Source: CAD feature listing. Evaluate the final solid. Frame: model axes, mm. Give positions to 0.01 mm unless a question says otherwise; leave off trailing zeros. Write each loop counter-clockwise with the first axis right and the second up, starting at its lowest first coordinate (ties: lowest second). Pieces come first, ordered by that corner, then holes. Notation, with made-up numbers: M 19.5,-12 L 78.5,-12 A23 cw 78.5,15 Z; hole C 17.25,43 d2. An arc over 180 degrees is marked long. Answer as a JSON object with one key per item and string values. Group by question number.
```python
from build123d import *

# Parameters (mm, degrees)
BASE_BLOCK_SKETCH_W         = 60
BASE_BLOCK_SKETCH_H         = 100
BASE_BLOCK_DEPTH            = 30
LOWER_CELL_POCKETS_SKETCH_W = 26
LOWER_CELL_POCKETS_SKETCH_H = 12
LOWER_CELL_POCKETS_DEPTH    = 66.574385243
UPPER_STEP_SKETCH_W         = 60
UPPER_STEP_SKETCH_H         = 57
UPPER_STEP_BOSS_DEPTH       = 20
UPPER_CELL_POCKETS_SKETCH_W = 26
UPPER_CELL_POCKETS_SKETCH_H = 16
UPPER_CELL_POCKETS_DEPTH    = 77.811457479
BACK_WALL_SLOTS_SKETCH_W    = 10.8
BACK_WALL_SLOTS_SKETCH_H    = 7
BACK_WALL_SLOTS_DEPTH       = 66.574385243


with BuildPart() as part:
    # Base Block Sketch → Base Block (new body)
    with BuildSketch(Plane.XY):
        Rectangle(BASE_BLOCK_SKETCH_W, BASE_BLOCK_SKETCH_H)
    extrude(amount=BASE_BLOCK_DEPTH)

    # Lower Cell Pockets Sketch → Lower Cell Pockets (cut, through all)
    with BuildSketch(Plane.XY.offset(30)):
        with Locations((14, 41)):
            Rectangle(LOWER_CELL_POCKETS_SKETCH_W, LOWER_CELL_POCKETS_SKETCH_H)
        Polygon((-21.788065722, 47), (-27, 47), (-27, 35), (-1, 35), (-1, 47), align=None)
    extrude(amount=-LOWER_CELL_POCKETS_DEPTH, mode=Mode.SUBTRACT)

    # Upper Step Sketch → Upper Step Boss (add)
    with BuildSketch(Plane.XY.offset(30)):
        with Locations((0, -21.5)):
            Rectangle(UPPER_STEP_SKETCH_W, UPPER_STEP_SKETCH_H)
    extrude(amount=UPPER_STEP_BOSS_DEPTH)

    # Upper Cell Pockets Sketch → Upper Cell Pockets (cut, through all)
    with BuildSketch(Plane.XY.offset(50)):
        with Locations((-14, -3)):
            Rectangle(UPPER_CELL_POCKETS_SKETCH_W, UPPER_CELL_POCKETS_SKETCH_H)
        with Locations((14, -3)):
            Rectangle(UPPER_CELL_POCKETS_SKETCH_W, UPPER_CELL_POCKETS_SKETCH_H)
        with Locations((14, -21)):
            Rectangle(UPPER_CELL_POCKETS_SKETCH_W, UPPER_CELL_POCKETS_SKETCH_H)
        with Locations((14, -39)):
            Rectangle(UPPER_CELL_POCKETS_SKETCH_W, UPPER_CELL_POCKETS_SKETCH_H)
        with Locations((-14, -21)):
            Rectangle(UPPER_CELL_POCKETS_SKETCH_W, UPPER_CELL_POCKETS_SKETCH_H)
        with Locations((-14, -39)):
            Rectangle(UPPER_CELL_POCKETS_SKETCH_W, UPPER_CELL_POCKETS_SKETCH_H)
    extrude(amount=-UPPER_CELL_POCKETS_DEPTH, mode=Mode.SUBTRACT)

    # Back Wall Slots Sketch → Back Wall Slots (cut, through all)
    with BuildSketch(Plane.XY.offset(30)):
        Polygon((27, 14), (16.2, 14), (16.2, 9), (25, 9), (27, 11), align=None)
        with Locations((0, 24.5)):
            Rectangle(BACK_WALL_SLOTS_SKETCH_W, BACK_WALL_SLOTS_SKETCH_H)
        Polygon((-16.2, 33), (-25, 33), (-27, 31), (-27, 28), (-16.2, 28), align=None)
        Polygon((25, 33), (16.2, 33), (16.2, 28), (27, 28), (27, 31), align=None)
        Polygon((-16.2, 14), (-27, 14), (-27, 11), (-25, 9), (-16.2, 9), align=None)
    extrude(amount=-BACK_WALL_SLOTS_DEPTH, mode=Mode.SUBTRACT)


solid = part.part
```
(1) Ray query, L1, parallel to Y at x = 5, z = 44.5; L2, parallel to Y at x = 10, z = 9.5; L3, parallel to X at y = -25, z = 19. Return the intervals inside material, ascending. Write a range as [from, to].
(2) Section B-B, the plane z = 34.5. Return loops of the section in (x, y).
(3) Section A-A, the plane y = 26.5. Return loops of the section in (x, z).
(4) Pull-direction query (X, two-part tool) for faces 1 (the flat face through (14, -13, 25)), 2 (the flat face through (22, 28, 15)), 3 (the flat face through (-30, -12, 19)), 4 (the flat face through (0, 50, 15)); classes: pulls with the +X half, pulls with the -X half, needs draft (parallel to the pull), parting line crosses it, or undercut.
(5) Section D-D, the plane x = -3.5. Return loops of the section in (y, z).
(6) Contact query for flat-ended pins moving along their axis: pin 1 Ø8 at (x, z) = (-16, 43) entering from +Y; pin 2 Ø10 at (x, y) = (-9, 16.5) entering from +Z. Output: stop coordinate, or through.
(7) Section C-C, the plane y = 2.5. Return loops of the section in (x, z).
Reported:
{
 "1": {"L1": "y = [-50, -47], [-31, -29], [-13, -11], [5, 7]", "L2": "y = [-50, -47], [-31, -29], [-13, -11], [5, 35], [47, 50]", "L3": "x = [-30, -27], [-1, 1], [27, 30]"},
 "2": {"outline": "M -30,-50 L 30,-50 L 30,7 L -30,7 Z; hole M -27,-47 L -1,-47 L -1,-31 L -27,-31 Z; hole M -27,-29 L -1,-29 L -1,-13 L -27,-13 Z; hole M -27,-11 L -1,-11 L -1,5 L -27,5 Z; hole M 1,-47 L 27,-47 L 27,-31 L 1,-31 Z; hole M 1,-29 L 27,-29 L 27,-13 L 1,-13 Z; hole M 1,-11 L 27,-11 L 27,5 L 1,5 Z"},
 "3": {"outline": "M -30,0 L -5.4,0 L -5.4,30 L -30,30 Z; M 5.4,0 L 30,0 L 30,30 L 5.4,30 Z"},
 "4": {"face 1": "undercut", "face 2": "undercut", "face 3": "pulls with the -X half", "face 4": "needs draft"},
 "5": {"outline": "M -50,0 L -47,0 L -47,50 L -50,50 Z; M -31,0 L -29,0 L -29,50 L -31,50 Z; M -13,0 L -11,0 L -11,50 L -13,50 Z; M 5,0 L 21,0 L 21,30 L 7,30 L 7,50 L 5,50 Z; M 28,0 L 35,0 L 35,30 L 28,30 Z; M 47,0 L 50,0 L 50,30 L 47,30 Z"},
 "6": {"pin 1": "stops at y = 7", "pin 2": "stops at z = 30"},
 "7": {"outline": "M -30,0 L -27,0 L -27,50 L -30,50 Z; M -1,0 L 1,0 L 1,50 L -1,50 Z; M 27,0 L 30,0 L 30,50 L 27,50 Z"}
}
